from build123d import *

# Parameters (mm, degrees)
BASE_PLATE_SKETCH_W           = 251
BASE_PLATE_SKETCH_H           = 160
BASE_PLATE_DEPTH              = 22
HOUSING_BLOCK_SKETCH_W        = 161
HOUSING_BLOCK_SKETCH_H        = 116
HOUSING_BLOCK_DEPTH           = 84
HOUSING_PROFILE_CUT_DEPTH     = 116
HOUSING_TRIM_CUT_SKETCH_W     = 38
HOUSING_TRIM_CUT_SKETCH_H     = 77
HOUSING_TRIM_CUT_DEPTH        = 200
MOUNTING_BOSSES_SKETCH_R      = 14
MOUNTING_BOSSES_DEPTH         = 12
MOUNTING_HOLES_SET_1_SKETCH_R = 8
MOUNTING_HOLES_SET_1_DEPTH    = 20
MOUNTING_HOLES_SET_2_SKETCH_R = 8
MOUNTING_HOLES_SET_2_DEPTH    = 20
HOUSING_POCKET_SKETCH_W       = 145
HOUSING_POCKET_SKETCH_H       = 100
HOUSING_POCKET_DEPTH          = 60
INNER_POCKET_DEPTH            = 40
POCKET_STEP_CUT_SKETCH_W      = 47.620155069
POCKET_STEP_CUT_SKETCH_H      = 77
POCKET_STEP_CUT_DEPTH         = 17
BEARING_HUB_54_SKETCH_R       = 27
BEARING_HUB_54_DEPTH          = 34
FRONT_START                   = 6
FRONT_BOSS_54_SKETCH_R        = 27
FRONT_BOSS_54_DEPTH           = 6
HUB_START                     = -6
HUB_RECESS_54_SKETCH_R        = 27
HUB_RECESS_54_DEPTH           = 6
SHAFT_BORE_22_SKETCH_R        = 11
SHAFT_BORE_22_DEPTH           = 33


with BuildPart() as part:
    # Base Plate Sketch → Base Plate (new body)
    with BuildSketch(Plane.XY):
        with Locations((125.5, 80)):
            Rectangle(BASE_PLATE_SKETCH_W, BASE_PLATE_SKETCH_H)
    extrude(amount=BASE_PLATE_DEPTH)

    # Housing Block Sketch → Housing Block (add)
    with BuildSketch(Plane.XY.offset(22)):
        with Locations((125.5, 80)):
            Rectangle(HOUSING_BLOCK_SKETCH_W, HOUSING_BLOCK_SKETCH_H)
    extrude(amount=HOUSING_BLOCK_DEPTH)

    # Housing Profile Cut Sketch → Housing Profile Cut (cut)
    with BuildSketch(Plane.XZ.offset(-22)):
        Polygon((85, 106), (45, 62), (45, 106), align=None)
    extrude(amount=-HOUSING_PROFILE_CUT_DEPTH, mode=Mode.SUBTRACT)

    # Housing Trim Cut Sketch → Housing Trim Cut (cut)
    with BuildSketch(Plane(origin=(-6.221719457, 0, 5.656108597), x_dir=(0.6726727939963125, 0, 0.7399400733959438), z_dir=(-0.7399400733959438, 0, 0.6726727939963125))):
        with Locations((105.378697775, 80)):
            Rectangle(HOUSING_TRIM_CUT_SKETCH_W, HOUSING_TRIM_CUT_SKETCH_H)
    extrude(amount=-HOUSING_TRIM_CUT_DEPTH, mode=Mode.SUBTRACT)

    # Mounting Bosses Sketch → Mounting Bosses (add)
    with BuildSketch(Plane.XY.offset(22)):
        with Locations((229, 122)):
            Circle(MOUNTING_BOSSES_SKETCH_R)
        with Locations((229, 38)):
            Circle(MOUNTING_BOSSES_SKETCH_R)
        with Locations((22, 38)):
            Circle(MOUNTING_BOSSES_SKETCH_R)
        with Locations((22, 122)):
            Circle(MOUNTING_BOSSES_SKETCH_R)
    extrude(amount=MOUNTING_BOSSES_DEPTH)

    # Mounting Holes Set 1 Sketch → Mounting Holes Set 1 (cut)
    with BuildSketch(Plane.XY.offset(22)):
        with Locations((22, 122)):
            Circle(MOUNTING_HOLES_SET_1_SKETCH_R)
        with Locations((22, 38)):
            Circle(MOUNTING_HOLES_SET_1_SKETCH_R)
        with Locations((229, 38)):
            Circle(MOUNTING_HOLES_SET_1_SKETCH_R)
        with Locations((229, 122)):
            Circle(MOUNTING_HOLES_SET_1_SKETCH_R)
    extrude(amount=-MOUNTING_HOLES_SET_1_DEPTH, mode=Mode.SUBTRACT)

    # Mounting Holes Set 2 Sketch → Mounting Holes Set 2 (cut)
    with BuildSketch(Plane.XY.offset(34)):
        with Locations((229, 122)):
            Circle(MOUNTING_HOLES_SET_2_SKETCH_R)
        with Locations((229, 38)):
            Circle(MOUNTING_HOLES_SET_2_SKETCH_R)
        with Locations((22, 38)):
            Circle(MOUNTING_HOLES_SET_2_SKETCH_R)
        with Locations((22, 122)):
            Circle(MOUNTING_HOLES_SET_2_SKETCH_R)
    extrude(amount=-MOUNTING_HOLES_SET_2_DEPTH, mode=Mode.SUBTRACT)

    # Housing Pocket Sketch → Housing Pocket (cut)
    with BuildSketch(Plane(origin=(0, 0, 0), x_dir=(-1, 0, 0), z_dir=(0, 0, -1))):
        with Locations((-125.5, 80)):
            Rectangle(HOUSING_POCKET_SKETCH_W, HOUSING_POCKET_SKETCH_H)
    extrude(amount=-HOUSING_POCKET_DEPTH, mode=Mode.SUBTRACT)

    # Inner Pocket Sketch → Inner Pocket (cut)
    with BuildSketch(Plane(origin=(0, 0, 60), x_dir=(-1, 0, 0), z_dir=(0, 0, -1))):
        Polygon((-198, 130), (-119.606684276, 130), (-119.606684276, 28.92459706), (-198, 30), align=None)
    extrude(amount=-INNER_POCKET_DEPTH, mode=Mode.SUBTRACT)

    # Pocket Step Cut Sketch → Pocket Step Cut (cut)
    with BuildSketch(Plane(origin=(83.666166146, 0, 92.032782761), x_dir=(-0.7399400733959437, 0, 0.6726727939963125), z_dir=(-0.6726727939963125, 0, -0.7399400733959437))):
        with Locations((-23.810077535, 80)):
            Rectangle(POCKET_STEP_CUT_SKETCH_W, POCKET_STEP_CUT_SKETCH_H)
    extrude(amount=-POCKET_STEP_CUT_DEPTH, mode=Mode.SUBTRACT)

    # Bearing Hub Ø54 Sketch → Bearing Hub Ø54 (add)
    with BuildSketch(Plane.XY.offset(106)):
        with Locations((145.5, 80)):
            Circle(BEARING_HUB_54_SKETCH_R)
    extrude(amount=-BEARING_HUB_54_DEPTH)

    # Front Boss Ø54 Sketch → Front Boss Ø54 (add)
    with BuildSketch(Plane.XY.offset(106).offset(FRONT_START)):
        with Locations((145.5, 80)):
            Circle(FRONT_BOSS_54_SKETCH_R)
    extrude(amount=-FRONT_BOSS_54_DEPTH)

    # Hub Recess Ø54 Sketch → Hub Recess Ø54 (cut)
    with BuildSketch(Plane(origin=(0, 0, 72), x_dir=(-1, 0, 0), z_dir=(0, 0, -1)).offset(HUB_START)):
        with Locations(Location((-145.5, 80, 0), (0, 0, 16.461230985))):
            Circle(HUB_RECESS_54_SKETCH_R)
    extrude(amount=HUB_RECESS_54_DEPTH, mode=Mode.SUBTRACT)

    # Shaft Bore Ø22 Sketch → Shaft Bore Ø22 (cut)
    with BuildSketch(Plane.XY.offset(112)):
        with Locations((145.5, 80)):
            Circle(SHAFT_BORE_22_SKETCH_R)
    extrude(amount=-SHAFT_BORE_22_DEPTH, mode=Mode.SUBTRACT)


solid = part.part
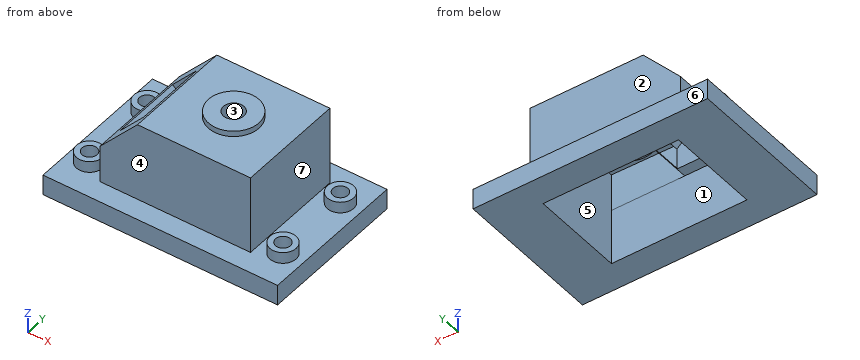
The model under review builds one solid part; all positions refer to its coordinate system, in mm. Face numbers are marked on the shaded views. A direction names the side the tool comes from. Round coordinates to 2 decimals unless told otherwise and drop trailing zeros. Loops run counter-clockwise (first coordinate to the right, second up) from the corner with the lowest first, then second, coordinate; pieces in that order, holes last. Notation, with made-up numbers: (71, 43.25) -> (100, 43.25) arc R14 cw to (100, 50.25) -> close; hole circle Ø3 at (24, 23.25). An arc over 180 degrees is marked (long way). Return JSON: item names as keys, results as strings.
(1) For the marked faces 1, 2, 3 and 4, list the 3-axis set-ups (+Z, -Z, +X, -X, +Y, -Y) from which the entire face can be reached by the end or side of a thin tool; tool diameter is ignored.
Solved:
{"face 1": "-Z", "face 2": "+Z, +X, -X, +Y", "face 3": "+Z", "face 4": "+Z, +X, -X, -Y"}
(2) Add section B-B on x = 65.5. Write out the cut boundary in (y, z).
Solved:
{"outline": "(0, 0) -> (30, 0) -> (30, 60) -> (41.5, 60) -> (41.5, 84.55) -> (22, 84.55) -> (22, 22) -> (0, 22) -> close; (118.5, 60) -> (130, 60) -> (130, 0) -> (160, 0) -> (160, 22) -> (138, 22) -> (138, 84.55) -> (118.5, 84.55) -> close"}
(3) Add section D-D on z = 15.5. Write out the cut boundary in (x, y), plus the area to 3 significant figures.
Solved:
{"outline": "(0, 0) -> (251, 0) -> (251, 160) -> (0, 160) -> close; hole circle Ø16 at (22, 38); hole circle Ø16 at (22, 122); hole (53, 30) -> (198, 30) -> (198, 130) -> (53, 130) -> close; hole circle Ø16 at (229, 38); hole circle Ø16 at (229, 122)", "area": "24,900 mm2"}
(4) For line 1 (Y direction, x = 229, z = 25); line 2 (Y direction, x = 22, z = 14); line 3 (Y direction, x = 197.5, z = 93), list the stretches that pass through material, from the lowest coordinate up.
Solved:
{"line 1": "24 to 30, 46 to 52, 108 to 114, 130 to 136", "line 2": "0 to 30, 46 to 114, 130 to 160", "line 3": "22 to 29.99, 130 to 138"}
(5) The part is to be moulded in two halves that separate along Y. For the marked faces 5, 6 and 7, say which applies: released by +Y, released by -Y, zero draft, split by the parting line, or undercut.
Solved:
{"face 5": "undercut", "face 6": "released by +Y", "face 7": "zero draft"}
(6) For pin 1 (17.5 mm diameter, centred on x = 145.5, y = 80, fed in from +Z); pin 2 (5 mm diameter, centred on x = 135, y = 128.5, fed in from +Z); pin 3 (5 mm diameter, centred on x = 45, z = 44, fed in from +Y); pin 4 (13 mm diameter, centred on x = 22, y = 122, fed in from -Z), all flat-tipped, find the tip position at first contact; note any pin that passes through.
Solved:
{"pin 1": "z = 79", "pin 2": "z = 106", "pin 3": "y = 138", "pin 4": "z = 0"}
(7) Add section A-A on z = 28. State how many separate pieces and enclosed holes the cut face has, plus the area to 3 significant figures.
Solved:
{"separate pieces": "5", "enclosed holes": "5", "area": "5,830 mm2"}
